Build history of the part. All positions in model axes, mm. A direction names the side the tool comes from. Give positions to 0.01 mm unless a question says otherwise; leave off trailing zeros. Order: outer loops, then holes, each group sorted by start corner. A loop starts at its lowest first (then second) coordinate and runs counter-clockwise, first axis right, second up. Notation, with made-up numbers: M 80,-24.75 L 90,-24.75 A37 cw 90,11.25 Z; hole C 64.25,12.25 d6. An arc over 180 degrees is marked long. Answer as CSV lines item,"result".
from build123d import *

# Parameters (mm, degrees)
SKETCH1_W                  = 120
SKETCH1_H                  = 160
BOSS_EXTRUDE1_DEPTH        = 15
CHAMFER1_SIZE              = 8
SKETCH2_R                  = 37.5
CUT_EXTRUDE1_DEPTH         = 23
SKETCH3_R                  = 1
CUT_EXTRUDE2_DEPTH         = 10
M5_TAPPED_HOLE1_D          = 4.2
SKETCH8_R                  = 3
CUT_EXTRUDE4_DEPTH         = 55
M8_TAPPED_HOLE1_D          = 6.8
SKETCH11_R                 = 2.5
CUT_EXTRUDE5_DEPTH         = 33
SKETCH12_R                 = 4
CUT_EXTRUDE6_DEPTH         = 6
SKETCH13_W                 = 3
SKETCH13_H                 = 40
BOSS_EXTRUDE2_DEPTH        = 15
CHAMFER2_SIZE              = 0.5
SKETCH14_R                 = 1.794169989
SKETCH14_R_2               = 1.756446965
CUT_EXTRUDE7_DEPTH         = 5
M5_TAPPED_HOLE2_AT_2_COUNT = 2
M5_TAPPED_HOLE2_AT_2_PITCH = 80
SKETCH16_R                 = 2.75
CUT_EXTRUDE8_DEPTH         = 55
SKETCH17_R                 = 6
CUT_EXTRUDE9_DEPTH         = 3


with BuildPart() as part:
    # Sketch1 → Boss-Extrude1 (new body)
    with BuildSketch(Plane(origin=(0, 0, 0), x_dir=(1, 0, 0), z_dir=(0, 1, 0))):
        Rectangle(SKETCH1_W, SKETCH1_H)
    extrude(amount=BOSS_EXTRUDE1_DEPTH)

    # Chamfer1
    chamfer1_edges = [part.edges().sort_by_distance(p)[0] for p in [
        (60, 7.5, 80),
        (-60, 7.5, 80),
        (-60, 7.5, -80),
        (60, 7.5, -80),
    ]]
    chamfer(chamfer1_edges, length=CHAMFER1_SIZE)

    # Sketch2 → Cut-Extrude1 (cut)
    with BuildSketch(Plane(origin=(0, 15, 0), x_dir=(1, 0, 0), z_dir=(0, 1, 0))):
        with Locations(Location((0, 0, 0), (0, 0, 270))):
            Circle(SKETCH2_R)
    extrude(amount=-CUT_EXTRUDE1_DEPTH, mode=Mode.SUBTRACT)

    # Sketch3 → Cut-Extrude2 (cut)
    with BuildSketch(Plane.XZ):
        with Locations(Location((-40, 25, 0), (0, 0, 270))):
            Circle(SKETCH3_R)
        with Locations(Location((40, 25, 0), (0, 0, 90))):
            Circle(SKETCH3_R)
        with Locations(Location((-40, -25, 0), (0, 0, 90))):
            Circle(SKETCH3_R)
        with Locations(Location((40, -25, 0), (0, 0, 270))):
            Circle(SKETCH3_R)
    extrude(amount=-CUT_EXTRUDE2_DEPTH, mode=Mode.SUBTRACT)

    # M5 Tapped Hole1 (through all)
    with Locations(Plane(origin=(-40, 0, 25), x_dir=(0, 0, -1), z_dir=(0, -1, 0))):
        with Locations((0, 0), (0, 80), (50, 80), (50, 0)):
            Hole(M5_TAPPED_HOLE1_D / 2)

    # Sketch8 → Cut-Extrude4 (cut)
    with BuildSketch(Plane.XZ):
        with Locations(Location((-47.5, 70, 0), (0, 0, 270))):
            Circle(SKETCH8_R)
        with Locations(Location((0, 70, 0), (0, 0, 270))):
            Circle(SKETCH8_R)
        with Locations(Location((47.5, 70, 0), (0, 0, 90))):
            Circle(SKETCH8_R)
        with Locations(Location((47.5, -70, 0), (0, 0, 270))):
            Circle(SKETCH8_R)
        with Locations(Location((0, -70, 0), (0, 0, 90))):
            Circle(SKETCH8_R)
        with Locations(Location((-47.5, -70, 0), (0, 0, 90))):
            Circle(SKETCH8_R)
    extrude(amount=-CUT_EXTRUDE4_DEPTH, mode=Mode.SUBTRACT)

    # M8 Tapped Hole1 (through all)
    with Locations(Plane(origin=(47.5, 0, -70), x_dir=(0, 0, -1), z_dir=(0, -1, 0))):
        with Locations((0, 0), (0, -47.5), (0, -95), (-140, -95), (-140, -47.5), (-140, 0)):
            Hole(M8_TAPPED_HOLE1_D / 2)

    # Sketch11 → Cut-Extrude5 (cut)
    with BuildSketch(Plane.XZ):
        with Locations(Location((-50, 0, 0), (0, 0, 270))):
            Circle(SKETCH11_R)
        with Locations(Location((50, 0, 0), (0, 0, 90))):
            Circle(SKETCH11_R)
    extrude(amount=-CUT_EXTRUDE5_DEPTH, mode=Mode.SUBTRACT)

    # Sketch12 → Cut-Extrude6 (cut)
    with BuildSketch(Plane(origin=(0, 15, 0), x_dir=(1, 0, 0), z_dir=(0, 1, 0))):
        with Locations(Location((-50, 0, 0), (0, 0, 270))):
            Circle(SKETCH12_R)
        with Locations(Location((50, 0, 0), (0, 0, 270))):
            Circle(SKETCH12_R)
    extrude(amount=-CUT_EXTRUDE6_DEPTH, mode=Mode.SUBTRACT)

    # Sketch13 → Boss-Extrude2 (add)
    with BuildSketch(Plane(origin=(0, 15, 0), x_dir=(1, 0, 0), z_dir=(0, 1, 0))):
        with Locations((-61.5, 0)):
            Rectangle(SKETCH13_W, SKETCH13_H)
        with Locations((61.5, 0)):
            Rectangle(SKETCH13_W, SKETCH13_H)
    extrude(amount=-BOSS_EXTRUDE2_DEPTH)

    # Chamfer2
    chamfer2_edges = [part.edges().sort_by_distance(p)[0] for p in [
        (63, 7.5, -20),
        (63, 7.5, 20),
        (-63, 7.5, -20),
        (-63, 7.5, 20),
    ]]
    chamfer(chamfer2_edges, length=CHAMFER2_SIZE)

    # Sketch14 → Cut-Extrude7 (cut)
    with BuildSketch(Plane(origin=(60, 0, 0), x_dir=(0, 0, -1), z_dir=(1, 0, 0))):
        with Locations((-40, 7.5)):
            Circle(SKETCH14_R)
        with Locations((40, 7.5)):
            Circle(SKETCH14_R_2)
    extrude(amount=-CUT_EXTRUDE7_DEPTH, mode=Mode.SUBTRACT)

    # Sketch15 → M5 Tapped Hole2 (revolve, cut)
    with BuildSketch(Plane(origin=(60, 7.5, 40), x_dir=(0, 0, -1), z_dir=(0, 1, 0))):
        Polygon((0, 0), (0, 13.6618073), (2.1, 12.4), (2.1, 0), align=None)
    m5_tapped_hole2 = revolve(axis=Axis((66.35, 7.5, 40), (-1, 0, 0)), mode=Mode.SUBTRACT)

    # M5 Tapped Hole2 at 2: M5 Tapped Hole2 ×2
    with Locations(*[(0, 0, -i * M5_TAPPED_HOLE2_AT_2_PITCH) for i in range(1, M5_TAPPED_HOLE2_AT_2_COUNT)]):
        add(m5_tapped_hole2, mode=Mode.SUBTRACT)

    # Mirror1: M5 Tapped Hole2 across plane
    add(m5_tapped_hole2.mirror(Plane(origin=(0, 0, 0), x_dir=(0, 0, 1), z_dir=(1, 0, 0))), mode=Mode.SUBTRACT)

    # Mirror1 copy 1 sketch → Mirror1 copy 1 (revolve, cut)
    with BuildSketch(Plane(origin=(-60, 7.5, -40), x_dir=(0, 0, -1), z_dir=(0, 1, 0))):
        Polygon((0, 0), (0, -13.6618073), (2.1, -12.4), (2.1, 0), align=None)
    revolve(axis=Axis((-66.35, 7.5, -40), (-1, 0, 0)), mode=Mode.SUBTRACT)

    # Sketch16 → Cut-Extrude8 (cut)
    with BuildSketch(Plane(origin=(0, 15, 0), x_dir=(1, 0, 0), z_dir=(0, 1, 0))):
        with Locations(Location((0, 45, 0), (0, 0, 270))):
            Circle(SKETCH16_R)
        with Locations(Location((45, 45, 0), (0, 0, 270))):
            Circle(SKETCH16_R)
        with Locations(Location((-45, 45, 0), (0, 0, 270))):
            Circle(SKETCH16_R)
        with Locations(Location((-45, -45, 0), (0, 0, 270))):
            Circle(SKETCH16_R)
        with Locations(Location((45, -45, 0), (0, 0, 270))):
            Circle(SKETCH16_R)
        with Locations(Location((0, -45, 0), (0, 0, 270))):
            Circle(SKETCH16_R)
    extrude(amount=-CUT_EXTRUDE8_DEPTH, mode=Mode.SUBTRACT)

    # Sketch17 → Cut-Extrude9 (cut)
    with BuildSketch(Plane(origin=(0, 15, 0), x_dir=(1, 0, 0), z_dir=(0, 1, 0))):
        with Locations(Location((-45, -45, 0), (0, 0, 270))):
            Circle(SKETCH17_R)
        with Locations(Location((0, -45, 0), (0, 0, 270))):
            Circle(SKETCH17_R)
        with Locations(Location((45, -45, 0), (0, 0, 270))):
            Circle(SKETCH17_R)
        with Locations(Location((0, 45, 0), (0, 0, 270))):
            Circle(SKETCH17_R)
        with Locations(Location((45, 45, 0), (0, 0, 270))):
            Circle(SKETCH17_R)
        with Locations(Location((-45, 45, 0), (0, 0, 270))):
            Circle(SKETCH17_R)
    extrude(amount=-CUT_EXTRUDE9_DEPTH, mode=Mode.SUBTRACT)


solid = part.part
Item 1: Band-saw the part on C-C (y = 3.5). State how many separate pieces and enclosed holes the cut face has, and give its area (3 significant figures).
Geometry says:
separate pieces,"1"
enclosed holes,"19"
area,"14,400 mm2"
Item 2: Pull direction X, two halves, no side cores. Call faces 6 (the flat face through (-63, 8, 0)), 7 (the cylindrical face through (50.87, 7.6, 69.56)), 8 (the flat face through (-15, 15, -37)): released by +X, released by -X, zero draft, split by the parting line, or undercut.
Geometry says:
face 6,"released by -X"
face 7,"undercut"
face 8,"zero draft"
Item 3: Band-saw the part on B-B (x = 23). Give the cut face in (y, z), and give its area (3 significant figures).
Geometry says:
outline,"M 0,-80 L 15,-80 L 15,-29.62 L 0,-29.62 Z; M 0,29.62 L 15,29.62 L 15,80 L 0,80 Z"
area,"1,510 mm2"
Item 4: Band-saw the part on D-D (z = 25). Give the cut face in (x, y).
Geometry says:
outline,"M -60,0 L -42.1,0 L -42.1,15 L -60,15 Z; M -37.9,0 L -27.95,0 L -27.95,15 L -37.9,15 Z; M 27.95,0 L 37.9,0 L 37.9,15 L 27.95,15 Z; M 42.1,0 L 60,0 L 60,15 L 42.1,15 Z"
Item 5: Probe line 1 along Z through (x, y) = (39, 7.5); line 2 along Z through (x, y) = (3, 7.5); line 3 along Z through (x, y) = (28, 7.75). List the from-to ranges inside material, lowest first. Write a range as from..to.
Geometry says:
line 1,"z = -80..-26.85, -23.15..23.15, 26.85..80"
line 2,"z = -80..-71.6, -68.4..-37.38, 37.38..68.4, 71.6..80"
line 3,"z = -80..-24.94, 24.94..80"
Item 6: 3-axis set-ups, long thin cutter, end or side, ignore diameter. For faces 1 (the flat face through (-60, 7, 46)), 2 (the flat face through (60, 7, 46)), 3 (the conical face through (-46.56, 7.39, 39.65)), 4 (the flat face through (-48, 12, -44)), 5 (the cylindrical face through (53.887, 6.081, -38.452)): which of +Z, -Z, +X, -X, +Y, -Y reach the whole face in a straight line?
Geometry says:
face 1,"+Z, -X, +Y, -Y"
face 2,"+Z, +X, +Y, -Y"
face 3,"-X"
face 4,"+Y"
face 5,"+X"
Item 7: Drop flat-ended pins along their axis: pin 1 (2.5 mm diameter, centred on y = 7.5, z = 40, fed in from -X); pin 2 (5.5 mm diameter, centred on y = 7.5, z = 40, fed in from -X); pin 3 (5 mm diameter, centred on x = -12.5, z = -53.5, fed in from -Y); pin 4 (3.5 mm diameter, centred on x = 2.5, z = 46, fed in from +Y). Give the stop position or say it passes through.
Geometry says:
pin 1,"stops at x = -47.09"
pin 2,"stops at x = -60"
pin 3,"stops at y = 0"
pin 4,"stops at y = 12"
Item 8: Band-saw the part on A-A (z = 0). Give the cut face in (x, y), and give its area (3 significant figures).
Geometry says:
outline,"M -63,0 L -52.5,0 L -52.5,9 L -54,9 L -54,15 L -63,15 Z; M -47.5,0 L -37.5,0 L -37.5,15 L -46,15 L -46,9 L -47.5,9 Z; M 37.5,0 L 47.5,0 L 47.5,9 L 46,9 L 46,15 L 37.5,15 Z; M 52.5,0 L 63,0 L 63,15 L 54,15 L 54,9 L 52.5,9 Z"
area,"579 mm2"
